```python
from build123d import *

# Parameters (mm, degrees)
F_110_X_110_X_5_1_DEPTH = 600
CUT_EXTRUDE_1_REACH     = 614.474


with BuildPart() as part:
    # Sketch1 → 方形管 110 X 110 X 5(1) (new body)
    with BuildSketch(Plane(origin=(0, 0, 0), x_dir=(0, 0, -1), z_dir=(1, 0, 0))):
        with BuildLine():
            Line((-45, -55), (45, -55))
            ThreePointArc((45, -55), (52.071067812, -52.071067812), (55, -45))
            Line((55, -45), (55, 45))
            ThreePointArc((55, 45), (52.071067812, 52.071067812), (45, 55))
            Line((45, 55), (-45, 55))
            ThreePointArc((-45, 55), (-52.071067812, 52.071067812), (-55, 45))
            Line((-55, 45), (-55, -45))
            ThreePointArc((-55, -45), (-52.071067812, -52.071067812), (-45, -55))
        make_face()
        with BuildLine():
            Line((-45, -50), (45, -50))
            ThreePointArc((45, -50), (48.535533906, -48.535533906), (50, -45))
            Line((50, -45), (50, 45))
            ThreePointArc((50, 45), (48.535533906, 48.535533906), (45, 50))
            Line((45, 50), (-45, 50))
            ThreePointArc((-45, 50), (-48.535533906, 48.535533906), (-50, 45))
            Line((-50, 45), (-50, -45))
            ThreePointArc((-50, -45), (-48.535533906, -48.535533906), (-45, -50))
        make_face(mode=Mode.SUBTRACT)
    extrude(amount=F_110_X_110_X_5_1_DEPTH)

    # 切除-拉伸1: up to this face of the body (flat: up to its plane)
    cut_extrude_1_end = Plane(part.part.faces().sort_by_distance((300, 0, -55))[0])
    # 草图2 → 切除-拉伸1 (cut, up to the picked face)
    with BuildSketch(Plane.XY.offset(55), mode=Mode.PRIVATE) as cut_extrude_1_sk1:
        Polygon((0, 148.583103171), (22.456015583, -55), (0, -55), align=None)
    cut_extrude_1_tool1 = split(extrude(cut_extrude_1_sk1.sketch, amount=-CUT_EXTRUDE_1_REACH, mode=Mode.PRIVATE), bisect_by=cut_extrude_1_end, keep=Keep.BOTH, mode=Mode.PRIVATE)
    # 草图2 → 切除-拉伸1 (cut, up to the picked face)
    with BuildSketch(Plane.XY.offset(55), mode=Mode.PRIVATE) as cut_extrude_1_sk2:
        Polygon((600, -274.46804857), (563.658380693, 55), (600, 55), align=None)
    cut_extrude_1_tool2 = split(extrude(cut_extrude_1_sk2.sketch, amount=-CUT_EXTRUDE_1_REACH, mode=Mode.PRIVATE), bisect_by=cut_extrude_1_end, keep=Keep.BOTH, mode=Mode.PRIVATE)
    add(cut_extrude_1_tool1.solids().sort_by(Axis((7.485339, 12.861034, 55), (0, 0, -1)))[0], mode=Mode.SUBTRACT)
    add(cut_extrude_1_tool2.solids().sort_by(Axis((587.886127, -54.822683, 55), (0, 0, -1)))[0], mode=Mode.SUBTRACT)


solid = part.part
```
Input: part model. Units: mm. Frame: model coordinates. A direction names the side the tool comes from. Round coordinates to 2 decimals unless told otherwise and drop trailing zeros. Loops run counter-clockwise (first coordinate to the right, second up) from the corner with the lowest first, then second, coordinate; pieces in that order, holes last. Notation, with made-up numbers: (17, -9.5) - (34, -9.5) arc R18 ccw to (34, 11.5) - close; hole circle Ø1 at (-26.5, 34). An arc over 180 degrees is marked (long way). One line per item, written item: value. Start each with the question number.
(1) Draft query along Z for faces 1 (the flat face through (289, -1, -55)), 2 (the flat face through (289, -1, -50)), 3 (the flat face through (283, 55, -1)). Return one class per face: +Z half, -Z half, draft (parallel to the pull), parting line (faces both ways), or undercut.
(2) Section B-B, the plane y = 27.5. Return loops of the section in (x, z).
(3) Section C-C, the plane x = 488. Return loops of the section in (y, z).
(4) Section A-A, the plane z = -33. Return loops of the section in (x, y).
(5) Ray query, line 1 (Y direction, x = 510, z = -45); line 2 (X direction, y = 50.5, z = 18.5). Return the intervals inside material, ascending. Write a range as [from, to].
(6) Contact query for a flat-ended pin moving along its axis: P1, Ø10, axis at y = 41, z = 30, coming from the -X side. Output: stop coordinate, or through.
(7) Access query for faces 4 (the flat face through (15.91, 4.33, -52.71)), 5 (the flat face through (289, 1, 50)). Directions: +Z, -Z, +X, -X, +Y, -Y. A direction counts if a zero-diameter tool reaches every point of the face in a straight line with its end or side. Return the directions, or none.
Results below:
1. face 1: -Z half
1. face 2: undercut
1. face 3: draft
2. outline: (13.36, -55) - (566.69, -55) - (566.69, -50) - (13.36, -50) - close; (13.36, 50) - (566.69, 50) - (566.69, 55) - (13.36, 55) - close
3. outline: (-55, -45) arc R10 ccw to (-45, -55) - (45, -55) arc R10 ccw to (55, -45) - (55, 45) arc R10 ccw to (45, 55) - (-45, 55) arc R10 ccw to (-55, 45) - close; hole (-50, -45) arc R5 ccw to (-45, -50) - (45, -50) arc R5 ccw to (50, -45) - (50, 45) arc R5 ccw to (45, 50) - (-45, 50) arc R5 ccw to (-50, 45) - close
4. outline: (10.32, 55) - (10.87, 50) - (564.21, 50) - (563.66, 55) - close; (21.9, -50) - (22.46, -55) - (575.79, -55) - (575.24, -50) - close
5. line 1: [-55, -50], [50, 55]
5. line 2: [10.82, 564.15]
6. P1: through
7. face 4: +Z, -Z, -X, -Y
7. face 5: +X, -X
